Check sheet for the modelled part. Datum: model origin and axes. Units: mm. Round coordinates to 2 decimals unless told otherwise and drop trailing zeros. Write each loop counter-clockwise with the first axis right and the second up, starting at its lowest first coordinate (ties: lowest second). Pieces come first, ordered by that corner, then holes. Notation, with made-up numbers: (-23.75, 58) -> (-11.75, 58) arc R11 cw to (-11.75, 70) -> close; hole circle Ø11 at (80, -31.75). An arc over 180 degrees is marked (long way). One line per item, written item: value. Start each with the question number.
```python
from build123d import *

# Parameters (mm, degrees)
SKETCH1_W           = 100
SKETCH1_H           = 30
BOSS_EXTRUDE1_DEPTH = 5
FILLET1_R           = 3
SKETCH3_R           = 5.5
CUT_EXTRUDE1_DEPTH  = 10


with BuildPart() as part:
    # Sketch1 → Boss-Extrude1 (new body)
    with BuildSketch(Plane(origin=(0, 0, 0), x_dir=(1, 0, 0), z_dir=(0, 1, 0))):
        Rectangle(SKETCH1_W, SKETCH1_H)
    extrude(amount=BOSS_EXTRUDE1_DEPTH)

    # Fillet1
    fillet1_edges = [part.edges().sort_by_distance(p)[0] for p in [
        (50, 2.5, 15),
        (-50, 2.5, 15),
        (-50, 2.5, -15),
        (50, 2.5, -15),
    ]]
    fillet(fillet1_edges, radius=FILLET1_R)

    # Sketch3 → Cut-Extrude1 (cut)
    with BuildSketch(Plane(origin=(0, 5, 0), x_dir=(1, 0, 0), z_dir=(0, 1, 0))):
        with Locations(Location((-40, 0, 0), (0, 0, 270))):
            Circle(SKETCH3_R)
        with Locations(Location((40, 0, 0), (0, 0, 270))):
            Circle(SKETCH3_R)
    extrude(amount=-CUT_EXTRUDE1_DEPTH, mode=Mode.SUBTRACT)


solid = part.part
```
1. Cross-section at A-A (z = 0). Record the cut outline in (x, y), plus the area to 3 significant figures.
2. Cross-section at C-C (x = 40). Record the cut outline in (y, z), plus the area to 3 significant figures.
3. Cross-section at B-B (y = 1.9). Record the cut outline in (x, z).
4. Material ranges on probe 1 along X at (y, z) = (2.4, 0); probe 2 along X at (y, z) = (2.6, 0.75); probe 3 along Z at (x, y) = (38.5, 4.5), recorded low to high.
5. Release check for a two-part mould opening along X. For faces 1 (the face through (-1, 0, 0)), 2 (the face through (-34.547, 2.535, -0.716)), 3 (the face through (45.453, 2.535, -0.716)), 4 (the face through (50, 2, 0)) record: +X half, -X half, draft (parallel to the pull), parting line (faces both ways), or undercut.
6. Depth check by flat-ended pin: pin 1 Ø14.5 at (x, z) = (-40, 0) entering from -Y. Enter the tip coordinate at first touch or a pass-through.
Working result:
1. outline: (-50, 0) -> (-45.5, 0) -> (-45.5, 5) -> (-50, 5) -> close; (-34.5, 0) -> (34.5, 0) -> (34.5, 5) -> (-34.5, 5) -> close; (45.5, 0) -> (50, 0) -> (50, 5) -> (45.5, 5) -> close
1. area: 390 mm^2
2. outline: (0, -15) -> (5, -15) -> (5, -5.5) -> (0, -5.5) -> close; (0, 5.5) -> (5, 5.5) -> (5, 15) -> (0, 15) -> close
2. area: 95.0 mm^2
3. outline: (-50, -12) arc R3 ccw to (-47, -15) -> (47, -15) arc R3 ccw to (50, -12) -> (50, 12) arc R3 ccw to (47, 15) -> (-47, 15) arc R3 ccw to (-50, 12) -> close; hole circle Ø11 at (-40, 0); hole circle Ø11 at (40, 0)
4. probe 1: x = -50 to -45.5, -34.5 to 34.5, 45.5 to 50
4. probe 2: x = -50 to -45.45, -34.55 to 34.55, 45.45 to 50
4. probe 3: z = -15 to -5.29, 5.29 to 15
5. face 1: draft
5. face 2: undercut
5. face 3: undercut
5. face 4: +X half
6. pin 1: stops at y = 0
